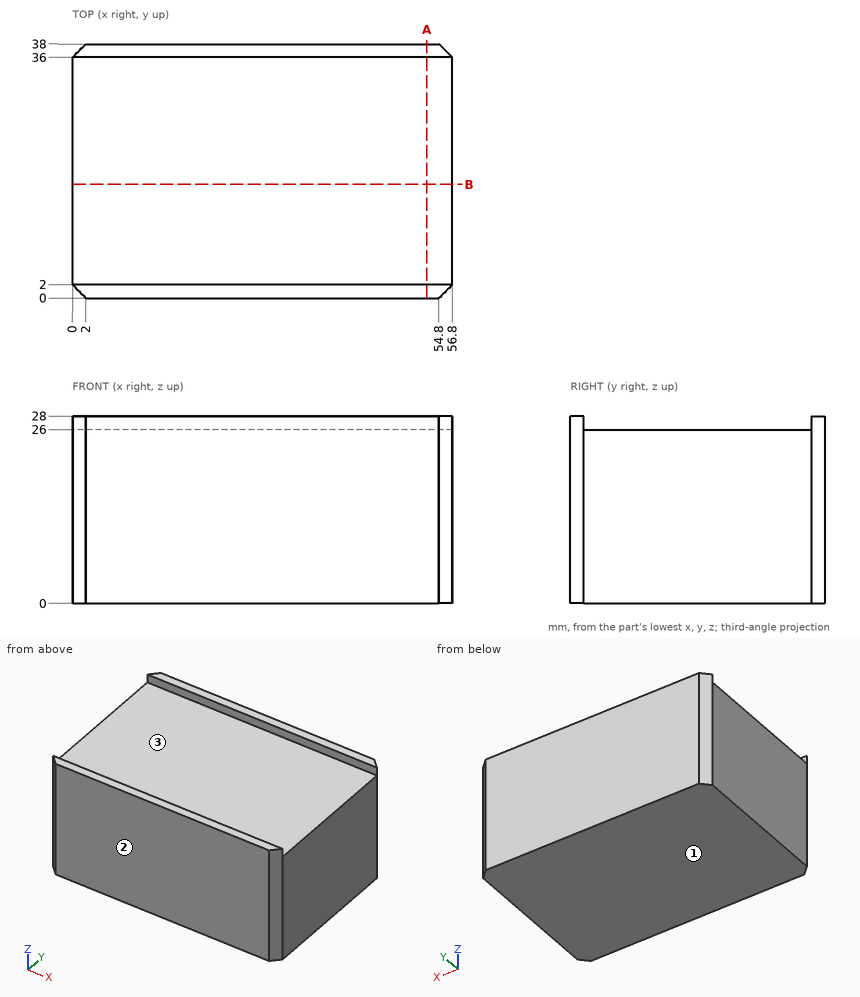
Drawing for the job (mm, zero at the part's lowest x, y, z). Round coordinates to 2 decimals unless told otherwise and drop trailing zeros. Loops run counter-clockwise (first coordinate to the right, second up) from the corner with the lowest first, then second, coordinate; pieces in that order, holes last. Notation, with made-up numbers: (15.25, 35.25) - (35.25, 35.25) arc R10 ccw to (35.25, 39.25) - close; hole circle Ø3 at (-22.75, -20.75). An arc over 180 degrees is marked (long way). Write each question's results on one line, items separated by ' | '.
(1) Saw through at A-A, the plane x = 53. List the corners of the cut face in (y, z), then the cut area to 3 significant figures.
Answer below:
outline: (0, 0) - (38, 0) - (38, 28) - (36, 28) - (36, 26) - (2, 26) - (2, 28) - (0, 28) - close | area: 996 mm^2
(2) Wall check: L1, parallel to Z at x = 7.5, y = 9.5. Give the ranges that are in metal, low to high.
Answer below:
L1: z = 0 to 26
(3) Mould opens along Y. For the marked faces 1, 2 and 3 say: released by +Y, released by -Y, zero draft, split by the parting line, or undercut.
Answer below:
face 1: zero draft | face 2: released by -Y | face 3: undercut
(4) Saw through at B-B, the plane y = 17. List the corners of the cut face in (x, z).
Answer below:
outline: (0, 0) - (56.8, 0) - (56.8, 26) - (0, 26) - close
